Model file for the job. Use its own axes, mm. A direction names the side the tool comes from. Coordinates: 2 decimals unless noted, no trailing zeros. Write each loop counter-clockwise with the first axis right and the second up, starting at its lowest first coordinate (ties: lowest second). Pieces come first, ordered by that corner, then holes. Notation, with made-up numbers: M 76.25,66.25 L 116.25,66.25 A19 cw 116.25,72.25 Z; hole C 17,-25 d9. An arc over 180 degrees is marked long. Put each result on its own line as item: value. Start each with the question number.
Q1. Cut at B-B (y = -7). Write the cut outline in (x, z), then the cut area to 3 significant figures.
Q2. Cut at A-A (x = -70). Write the cut outline in (y, z).
Q3. Drop flat-ended pins along their axis: pin 1 (4 mm diameter, centred on x = 60, z = 9.5, fed in from -Y); pin 2 (4 mm diameter, centred on x = 1, z = 7, fed in from +Y); pin 3 (9 mm diameter, centred on x = -70, z = 9.5, fed in from -Y); pin 4 (1 mm diameter, centred on x = 25, y = -11.5, fed in from +Z). Give the stop position or say it passes through.
Q4. Cut at C-C (x = 35.5). Write the cut outline in (y, z), then the cut area to 4 significant figures.
Q5. Which spindle directions (+Z, -Z, +X, -X, +Y, -Y) get a long thin tool onto all of the face, cutting with end or side? Do faces 1 (the flat face through (2.5, 10, 10)), 2 (the cylindrical face through (-61.65, -5.38, 9.43)), 3 (the flat face through (1, -10.5, 12)), 4 (the flat face through (-1, 1, 19)). Say none if no direction does.
Q6. Pull direction Z, two halves, no side cores. Call faces 5 (the flat face through (-1, 0, 0)), 6 (the cylindrical face through (66.7, 4.4, 9.4)), 7 (the flat face through (-42, 12.5, 9)): pulls with the +Z half, pulls with the -Z half, needs draft (parallel to the pull), parting line crosses it, or undercut.
Q7. Drill centre lines: line 1 along X through (y, z) = (6.5, 9.5); line 2 along X through (y, z) = (8.75, 11); line 3 along Y through (x, z) = (75, 11). Where is each one in solid material? Low to high.
```python
from build123d import *

# Parameters (mm, degrees)
SKETCH_1_W                   = 160
SKETCH_1_H                   = 25
EXTRUDE_1_DEPTH              = 19
SKETCH_2_W                   = 160
SKETCH_2_H                   = 15
CUT_EXTRUDE_1_DEPTH          = 2
HOLE_WIZARD_M4_1_D           = 3.3
HOLE_WIZARD_M4_1_DEPTH       = 10.1
HOLE_WIZARD_M4_1_TIP         = 0.991420021
HOLE_WIZARD_M6_1_D           = 6.6
HOLE_WIZARD_M6_1_CBORE_D     = 11
HOLE_WIZARD_M6_1_CBORE_DEPTH = 6.5
SKETCH_7_W                   = 5
SKETCH_7_H                   = 5
CUT_EXTRUDE_2_DEPTH          = 84.170006613
SKETCH_10_W                  = 2
SKETCH_10_H                  = 2
CUT_EXTRUDE_3_DEPTH          = 162.608322805
CHAMFER_1_SIZE               = 0.5
HOLE_WIZARD_M3_1_D           = 2.5


with BuildPart() as part:
    # 草图1 → 凸台-拉伸1 (new body)
    with BuildSketch(Plane.XY):
        Rectangle(SKETCH_1_W, SKETCH_1_H)
    extrude(amount=EXTRUDE_1_DEPTH)

    # 草图2 → 切除-拉伸1 (cut)
    with BuildSketch(Plane.XZ.offset(12.5)):
        with Locations((0, 9.5)):
            Rectangle(SKETCH_2_W, SKETCH_2_H)
    extrude(amount=-CUT_EXTRUDE_1_DEPTH, mode=Mode.SUBTRACT)

    # M4 螺纹孔1
    with Locations(Plane(origin=(0, -10.5, 0), x_dir=(-1, 0, 0), z_dir=(0, -1, 0))):
        with Locations((-60, -9.5), (0, -9.5), (60, -9.5)):
            Hole(HOLE_WIZARD_M4_1_D / 2, depth=HOLE_WIZARD_M4_1_DEPTH)
            with Locations((0, 0, -(HOLE_WIZARD_M4_1_DEPTH + HOLE_WIZARD_M4_1_TIP / 2))):  # 118° drill point
                Cone(0, HOLE_WIZARD_M4_1_D / 2, HOLE_WIZARD_M4_1_TIP, mode=Mode.SUBTRACT)

    # M6 六角凹头螺钉的柱形沉头孔1 (through all)
    with Locations(Plane(origin=(0, -10.5, 0), x_dir=(-1, 0, 0), z_dir=(0, -1, 0))):
        with Locations((-70, -9.5), (70, -9.5)):
            CounterBoreHole(HOLE_WIZARD_M6_1_D / 2, HOLE_WIZARD_M6_1_CBORE_D / 2, HOLE_WIZARD_M6_1_CBORE_DEPTH)

    # 草图7 → 切除-拉伸2 (cut, through all)
    with BuildSketch(Plane.XY.offset(19)):
        with Locations((0, 10)):
            Rectangle(SKETCH_7_W, SKETCH_7_H)
    extrude(amount=-CUT_EXTRUDE_2_DEPTH, mode=Mode.SUBTRACT)

    # 草图10 → 切除-拉伸3 (cut, through all)
    with BuildSketch(Plane(origin=(80, 0, 0), x_dir=(0, 0, -1), z_dir=(1, 0, 0))):
        with Locations((-18, -11.5)):
            Rectangle(SKETCH_10_W, SKETCH_10_H)
    extrude(amount=-CUT_EXTRUDE_3_DEPTH, mode=Mode.SUBTRACT)

    # 倒角1
    chamfer_1_edges = [part.edges().sort_by_distance(p)[0] for p in [
        (-80, 1, 19),
        (80, -12.5, 1),
        (-80, -12.5, 1),
        (80, -10.5, 10.5),
        (80, -11.5, 2),
        (-80, -10.5, 10.5),
        (-80, -11.5, 2),
        (0, -12.5, 0),
        (-80, 0, 0),
        (41.25, 12.5, 0),
        (80, 0, 0),
        (-41.25, 12.5, 0),
        (-41.25, 12.5, 19),
        (41.25, 12.5, 19),
        (-80, 12.5, 9.5),
        (80, 1, 19),
        (80, 12.5, 9.5),
        (0, -10.5, 19),
    ]]
    chamfer(chamfer_1_edges, length=CHAMFER_1_SIZE)

    # M3 螺纹孔1 (through all)
    with Locations(Plane.XY.offset(19)):
        with Locations((75, -0.5), (-75, -0.5)):
            Hole(HOLE_WIZARD_M3_1_D / 2)


solid = part.part
```
Computed values:
1. outline: M -80,0.5 L -79.5,0 L 79.5,0 L 80,0.5 L 80,18.5 L 79.5,19 L -79.5,19 L -80,18.5 Z; hole C -70,9.5 d11; hole C -60,9.5 d3.3; hole C 0,9.5 d3.3; hole C 60,9.5 d3.3; hole C 70,9.5 d11
1. area: 2,820 mm2
2. outline: M -12.5,0.5 L -12,0 L 12,0 L 12.5,0.5 L 12.5,6.2 L -4,6.2 L -4,4 L -10.5,4 L -10.5,2 L -12.5,2 Z; M -10.5,15 L -4,15 L -4,12.8 L 12.5,12.8 L 12.5,18.5 L 12,19 L -10,19 L -10.5,18.5 Z
3. pin 1: y = -10.5
3. pin 2: y = 12.5
3. pin 3: y = -4
3. pin 4: z = 2
4. outline: M -12.5,0.5 L -12,0 L 12,0 L 12.5,0.5 L 12.5,18.5 L 12,19 L -10,19 L -10.5,18.5 L -10.5,2 L -12.5,2 Z
4. area: 440.5 mm2
5. face 1: +Z, -Z, +Y
5. face 2: -Y
5. face 3: +Z, +X, -X, -Y
5. face 4: +Z, +X, -X, +Y, -Y
6. face 5: pulls with the -Z half
6. face 6: undercut
6. face 7: needs draft
7. line 1: -80 to -73.3, -66.7 to 66.7, 73.3 to 80
7. line 2: -80 to -72.94, -67.06 to -2.5, 2.5 to 67.06, 72.94 to 80
7. line 3: -4 to -1.75, 0.75 to 12.5
